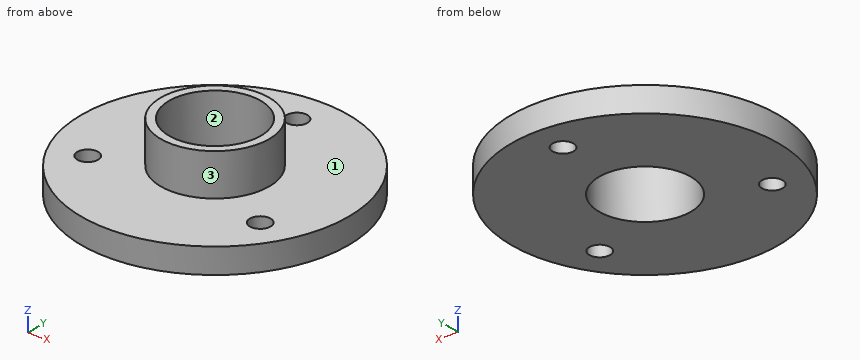
```python
from build123d import *

# Parameters (mm, degrees)
SKETCH1_R             = 16
BOSS_EXTRUDE1_DEPTH   = 3
SKETCH2_R             = 6.5
BOSS_EXTRUDE2_DEPTH   = 5
SKETCH3_R             = 5.5
CUT_EXTRUDE1_DEPTH    = 22
SKETCH4_R             = 1
CUT_EXTRUDE2_DEPTH    = 10
M3_TAPPED_HOLE1_D     = 2.5
M3_TAPPED_HOLE1_DEPTH = 8


with BuildPart() as part:
    # Sketch1 → Boss-Extrude1 (new body)
    with BuildSketch(Plane.XY):
        Circle(SKETCH1_R)
    extrude(amount=BOSS_EXTRUDE1_DEPTH)

    # Sketch2 → Boss-Extrude2 (add)
    with BuildSketch(Plane.XY.offset(3)):
        Circle(SKETCH2_R)
    extrude(amount=BOSS_EXTRUDE2_DEPTH)

    # Sketch3 → Cut-Extrude1 (cut)
    with BuildSketch(Plane(origin=(0, 0, 0), x_dir=(-1, 0, 0), z_dir=(0, 0, -1))):
        Circle(SKETCH3_R)
    extrude(amount=-CUT_EXTRUDE1_DEPTH, mode=Mode.SUBTRACT)

    # Sketch4 → Cut-Extrude2 (cut)
    with BuildSketch(Plane(origin=(0, 0, 0), x_dir=(-1, 0, 0), z_dir=(0, 0, -1))):
        with Locations((0, 12)):
            Circle(SKETCH4_R)
        with Locations((10.392304845, -6)):
            Circle(SKETCH4_R)
        with Locations((-10.392304845, -6)):
            Circle(SKETCH4_R)
    extrude(amount=-CUT_EXTRUDE2_DEPTH, mode=Mode.SUBTRACT)

    # M3 Tapped Hole1
    with Locations(Plane(origin=(0, 0, 0), x_dir=(-1, 0, 0), z_dir=(0, 0, -1))):
        with Locations((0, 12), (10.392304845, -6), (-10.392304845, -6)):
            Hole(M3_TAPPED_HOLE1_D / 2, depth=M3_TAPPED_HOLE1_DEPTH)


solid = part.part
```
Verification items for the finished model (mm, model axes). Face numbers are marked on the shaded views. Coordinates: 2 decimals unless noted, no trailing zeros. Write each loop counter-clockwise with the first axis right and the second up, starting at its lowest first coordinate (ties: lowest second). Pieces come first, ordered by that corner, then holes. Notation, with made-up numbers: M 87,79 L 110,79 A13 cw 110,98 Z; hole C -12,43 d7. An arc over 180 degrees is marked long. Answer as a JSON object with one key per item and string values. Group by question number.
(1) Material ranges on line 1 (Y direction, x = -0.5, z = 0.5); line 2 (Y direction, x = 0, z = 4); line 3 (Z direction, x = 14.5, y = -6), recorded low to high.
(2) Cross-section at A-A, the plane y = 0. Record the cut outline in (x, z).
(3) Cross-section at C-C, the plane y = -6. Record the cut outline in (x, z).
(4) Gauge pin test, flat ends, axial feed: pin 1 (3 mm diameter, centred on x = -7, y = -4.5, fed in from +Z); pin 2 (3 mm diameter, centred on y = 2.5, z = 2, fed in from -X); pin 3 (1 mm diameter, centred on x = -7, z = 2, fed in from -Y). Record the tip position at first contact, or that the pin passes through.
(5) Cross-section at D-D, the plane z = 5. Record the cut outline in (x, y), and give its area (3 significant figures).
(6) Release check for a two-part mould opening along X. For the marked faces 1, 2 and 3 record: +X half, -X half, draft (parallel to the pull), parting line (faces both ways), or undercut.
(7) Cross-section at B-B, the plane x = 0. Record the cut outline in (y, z), and give its area (3 significant figures).
Reply:
{
 "1": {"line 1": "-15.99 to -5.48, 5.48 to 10.85, 13.15 to 15.99", "line 2": "-6.5 to -5.5, 5.5 to 6.5", "line 3": "0 to 3"},
 "2": {"outline": "M -16,0 L -5.5,0 L -5.5,8 L -6.5,8 L -6.5,3 L -16,3 Z; M 5.5,0 L 16,0 L 16,3 L 6.5,3 L 6.5,8 L 5.5,8 Z"},
 "3": {"outline": "M -14.83,0 L -11.64,0 L -11.64,3 L -14.83,3 Z; M -9.14,0 L 9.14,0 L 9.14,3 L 2.5,3 L 2.5,8 L -2.5,8 L -2.5,3 L -9.14,3 Z; M 11.64,0 L 14.83,0 L 14.83,3 L 11.64,3 Z"},
 "4": {"pin 1": "z = 3", "pin 2": "x = -15.97", "pin 3": "y = -14.62"},
 "5": {"outline": "C 0,0 d13; hole C 0,0 d11", "area": "37.7 mm²"},
 "6": {"face 1": "draft", "face 2": "undercut", "face 3": "parting line"},
 "7": {"outline": "M -16,0 L -5.5,0 L -5.5,8 L -6.5,8 L -6.5,3 L -16,3 Z; M 5.5,0 L 10.75,0 L 10.75,3 L 6.5,3 L 6.5,8 L 5.5,8 Z; M 13.25,0 L 16,0 L 16,3 L 13.25,3 Z", "area": "65.5 mm²"}
}
